The figure shows three views and two pictorial views of one solid part (mm, origin at its lowest corner). Answer the questions. A direction names the side the tool comes from. Coordinates: 2 decimals unless noted, no trailing zeros. Order: outer loops, then holes, each group sorted by start corner. A loop starts at its lowest first (then second) coordinate and runs counter-clockwise, first axis right, second up. Notation, with made-up numbers: (85, 19) -> (97, 19) arc R22 ccw to (97, 37) -> close; hole circle Ø9 at (57, 86.25). An arc over 180 degrees is marked (long way). Return JSON: item names as keys, results as strings.
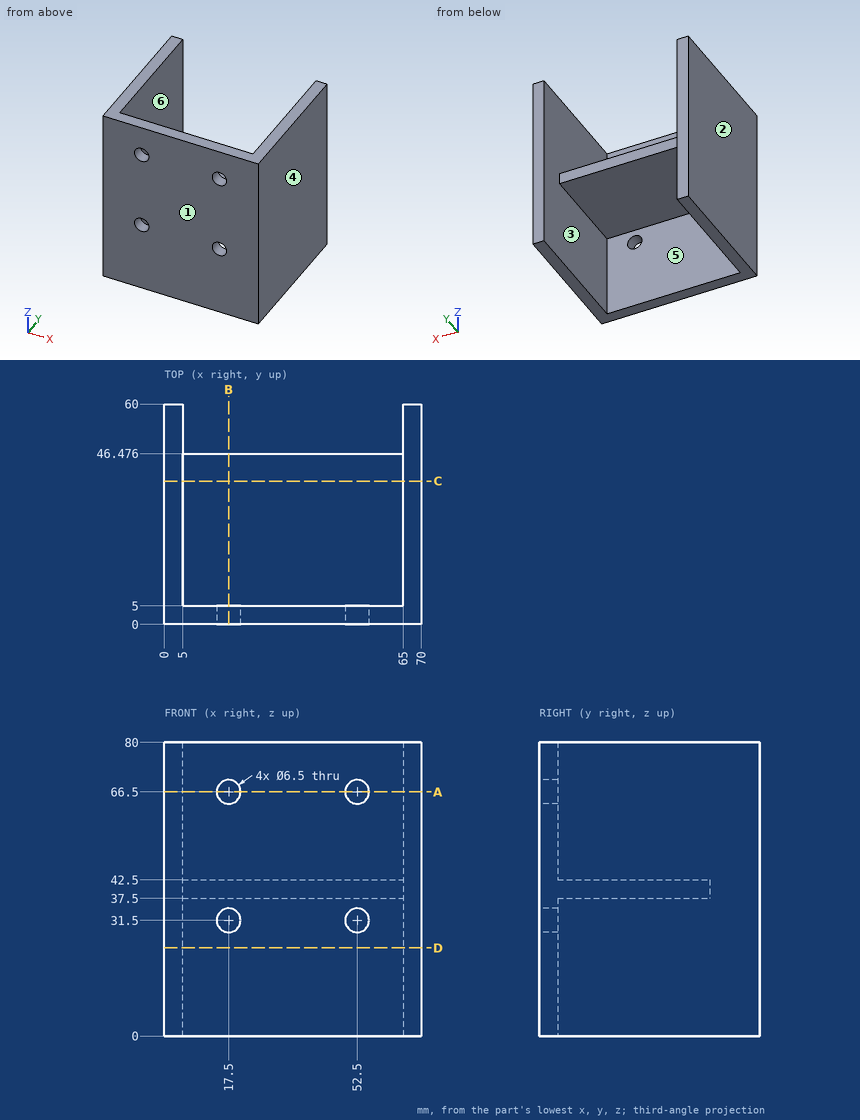
Item 1: Find the intervals of material crossed by probe 1 along Z at (x, y) = (52.5, 4.05); probe 2 along X at (y, z) = (3, 66); probe 3 along X at (y, z) = (8.5, 54), in increasing order.
Answer list:
{"probe 1": "0 to 28.25, 34.75 to 63.25, 69.75 to 80", "probe 2": "0 to 14.29, 20.71 to 49.29, 55.71 to 70", "probe 3": "0 to 5, 65 to 70"}
Item 2: The part is cut by section B-B on x = 17.5. Determine the outline of the cut face in (y, z).
Answer list:
{"outline": "(0, 0) -> (5, 0) -> (5, 28.25) -> (0, 28.25) -> close; (0, 34.75) -> (5, 34.75) -> (5, 37.5) -> (46.48, 37.5) -> (46.48, 42.5) -> (5, 42.5) -> (5, 63.25) -> (0, 63.25) -> close; (0, 69.75) -> (5, 69.75) -> (5, 80) -> (0, 80) -> close"}
Item 3: Flat-ended cylindrical pins translate along their axes: pin 1 (5 mm diameter, centred on x = 17.5, z = 31.5, fed in from -Y); pin 2 (5 mm diameter, centred on x = 43.5, y = 47.5, fed in from +Z); pin 3 (11 mm diameter, centred on x = 22, z = 70.5, fed in from +Y); pin 4 (2.5 mm diameter, centred on x = 40.5, z = 39, fed in from +Y). Find the tip coordinate at first contact, or state that the pin passes through.
Answer list:
{"pin 1": "through", "pin 2": "z = 42.5", "pin 3": "y = 5", "pin 4": "y = 46.48"}
Item 4: The part is cut by section D-D on z = 24. Determine the outline of the cut face in (x, y), plus the area to 3 significant figures.
Answer list:
{"outline": "(0, 0) -> (70, 0) -> (70, 60) -> (65, 60) -> (65, 5) -> (5, 5) -> (5, 60) -> (0, 60) -> close", "area": "900 mm2"}
Item 5: The part is cut by section A-A on z = 66.5. Determine the outline of the cut face in (x, y).
Answer list:
{"outline": "(0, 0) -> (14.25, 0) -> (14.25, 5) -> (5, 5) -> (5, 60) -> (0, 60) -> close; (20.75, 0) -> (49.25, 0) -> (49.25, 5) -> (20.75, 5) -> close; (55.75, 0) -> (70, 0) -> (70, 60) -> (65, 60) -> (65, 5) -> (55.75, 5) -> close"}
Item 6: Which of the six approach directions +Z, -Z, +X, -X, +Y, -Y give full straight-line access (tool end or side, diameter ignored) to the marked faces 4, 5 and 6?
Answer list:
{"face 4": "+Z, -Z, +X, +Y, -Y", "face 5": "-Z, +Y", "face 6": "+Y"}
Item 7: The part is cut by section C-C on y = 39. Determine the outline of the cut face in (x, z).
Answer list:
{"outline": "(0, 0) -> (5, 0) -> (5, 37.5) -> (65, 37.5) -> (65, 0) -> (70, 0) -> (70, 80) -> (65, 80) -> (65, 42.5) -> (5, 42.5) -> (5, 80) -> (0, 80) -> close"}
Item 8: Determine the mould class of the marked faces 1, 2 and 3 for opening direction X: pulls with the +X half, pulls with the -X half, needs draft (parallel to the pull), parting line crosses it, or undercut.
Answer list:
{"face 1": "needs draft", "face 2": "pulls with the -X half", "face 3": "undercut"}
